from build123d import *

# Parameters (mm, degrees)
BASE_PROFILE_20MM_DEPTH   = 20
A_FRAME_BODY_200MM_DEPTH  = 200
FRAME_WINDOW_1_SKETCH_W   = 124.025088206
FRAME_WINDOW_1_SKETCH_H   = 160
FRAME_WINDOW_1_CUT_DEPTH  = 30
FRAME_WINDOW_2_SKETCH_W   = 43.365918468
FRAME_WINDOW_2_SKETCH_H   = 160
FRAME_WINDOW_2_CUT_DEPTH  = 30
THROUGH_OPENING_SKETCH_W  = 51.957421724
THROUGH_OPENING_SKETCH_H  = 25.341390787
THROUGH_OPENING_CUT_DEPTH = 200
WEB_BOSS_30MM_DEPTH       = 30
HUB_BOSS_30MM_DEPTH       = 30
HUB_BORE_SKETCH_R         = 25
HUB_BORE_CUT_DEPTH        = 120


with BuildPart() as part:
    # Base Profile Sketch → Base Profile 20mm (new body)
    with BuildSketch(Plane.XY):
        with BuildLine():
            Line((0, 200), (0, 0))
            Line((0, 0), (200, 0))
            Line((200, 0), (200, 20))
            Line((200, 20), (130, 20))
            ThreePointArc((130, 20), (122.928932188, 22.928932188), (120, 30))
            Line((120, 30), (120, 160))
            Line((120, 160), (120, 170))
            ThreePointArc((120, 170), (122.928932188, 177.071067812), (130, 180))
            Line((130, 180), (200, 180))
            Line((200, 180), (200, 200))
            Line((200, 200), (0, 200))
        make_face()
    extrude(amount=BASE_PROFILE_20MM_DEPTH)

    # Frame Profile Sketch → A-Frame Body 200mm (add)
    with BuildSketch(Plane.XZ):
        Polygon((120.794177907, 115.439301395), (94.123171193, 115.439301395), (91.530156651, 115.439301395), (48.56020139, 115.439301395), (0, 20), (24.280100695, 20), (59.946420611, 90.097910608), (111.903842335, 90.097910608), (174.506621983, 20), (200, 20), align=None)
    extrude(amount=-A_FRAME_BODY_200MM_DEPTH)

    # Frame Window 1 Sketch → Frame Window 1 Cut (cut)
    with BuildSketch(Plane(origin=(128.259685241, 0, 106.443715141), x_dir=(0.6386274199814919, 0, -0.7695160936899132), z_dir=(0.7695160936899134, 0, 0.6386274199814919))):
        with Locations((50.32261802, 100)):
            Rectangle(FRAME_WINDOW_1_SKETCH_W, FRAME_WINDOW_1_SKETCH_H)
    extrude(amount=-FRAME_WINDOW_1_CUT_DEPTH, mode=Mode.SUBTRACT)

    # Frame Window 2 Sketch → Frame Window 2 Cut (cut)
    with BuildSketch(Plane.XY.offset(115.439301395)):
        with Locations((99.111218673, 100)):
            Rectangle(FRAME_WINDOW_2_SKETCH_W, FRAME_WINDOW_2_SKETCH_H)
    extrude(amount=-FRAME_WINDOW_2_CUT_DEPTH, mode=Mode.SUBTRACT)

    # Through Opening Sketch → Through Opening Cut (cut)
    with BuildSketch(Plane.XZ):
        with Locations((85.925131473, 102.768606002)):
            Rectangle(THROUGH_OPENING_SKETCH_W, THROUGH_OPENING_SKETCH_H)
    extrude(amount=-THROUGH_OPENING_CUT_DEPTH, mode=Mode.SUBTRACT)

    # Web Sketch → Web Boss 30mm (add)
    with BuildSketch(Plane.XY.offset(115.439301395)):
        with BuildLine():
            Line((48.56020139, 200), (120.794177907, 200))
            Line((120.794177907, 200), (120.794177907, 180))
            Line((120.794177907, 180), (97.556604563, 180))
            ThreePointArc((97.556604563, 180), (90.485536751, 177.071067812), (87.556604563, 170))
            Line((87.556604563, 170), (87.556604563, 30))
            ThreePointArc((87.556604563, 30), (90.485536751, 22.928932188), (97.556604563, 20))
            Line((97.556604563, 20), (120.794177907, 20))
            Line((120.794177907, 20), (120.794177907, 0))
            Line((120.794177907, 0), (48.56020139, 0))
            Line((48.56020139, 0), (48.56020139, 200))
        make_face()
    extrude(amount=-WEB_BOSS_30MM_DEPTH)

    # Hub Boss Sketch → Hub Boss 30mm (add)
    with BuildSketch(Plane.XY.offset(115.439301395)):
        with BuildLine():
            Line((87.556604563, 145), (87.556604563, 55))
            ThreePointArc((87.556604563, 55), (132.556604563, 100), (87.556604563, 145))
        make_face()
    extrude(amount=-HUB_BOSS_30MM_DEPTH)

    # Hub Bore Sketch → Hub Bore Cut (cut)
    with BuildSketch(Plane.XY.offset(115.439301395)):
        with Locations((87.556604563, 100)):
            Circle(HUB_BORE_SKETCH_R)
    extrude(amount=-HUB_BORE_CUT_DEPTH, mode=Mode.SUBTRACT)


solid = part.part
Design review of the part built by this model. Coordinates are the model's own, in mm. A direction names the side the tool comes from. Give positions to 0.01 mm unless a question says otherwise; leave off trailing zeros. Order: outer loops, then holes, each group sorted by start corner. A loop starts at its lowest first (then second) coordinate and runs counter-clockwise, first axis right, second up.
1. Tool access review of faces 5 (the cylindrical face through (122.85, 176.99, 9.86)), 6 (the flat face through (120, 99, 10)), 7 (the cylindrical face through (67.717, 84.788, 100.649)), 8 (the flat face through (149, 180, 49)), 9 (the flat face through (121, 0, 84)): name each direction out of +Z, -Z, +X, -X, +Y, -Y from which nothing blocks a thin tool from reaching the whole face with its end or side.
Solution:
face 5: +Z, -Z, +X
face 6: -Z, +X
face 7: +Z, -Z
face 8: +Z, +X
face 9: +Z, -Z, +X, -X, -Y
2. To check wall thickness, follow L1, parallel to Z at x = 75, y = 10; L2, parallel to Y at x = 89, z = 87; L3, parallel to Y at x = 104.5, z = 14. State the ranges of each line that lie inside material, in increasing order.
Solution:
L1: z = 0 to 20, 85.44 to 115.44
L2: y = 0 to 24.82, 55.02 to 75.04, 124.96 to 144.98, 175.18 to 200
L3: y = 0 to 81.62, 118.38 to 200
3. Add section B-B, the plane x = 183.5. State the section outline as (y, z) points, then the cut area to 3 significant figures.
Solution:
outline: (0, 0) - (20, 0) - (20, 39.88) - (0, 39.88) - close; (180, 0) - (200, 0) - (200, 39.88) - (180, 39.88) - close
area: 1,600 mm2
4. Add section C-C, the plane y = 17. State the section outline as (x, z) points.
Solution:
outline: (0, 0) - (200, 0) - (200, 20) - (120.79, 115.44) - (48.56, 115.44) - (0, 20) - close; hole (24.28, 20) - (174.51, 20) - (116.06, 85.44) - (57.58, 85.44) - close
5. Mouldability with a two-part tool opening along Y and no side actions: class faces 1 (the flat face through (121, 200, 84)), 2 (the flat face through (54, 101, 0)), 3 (the flat face through (149, 20, 49)), 4 (the cylindrical face through (132.546, 99.01, 100.649)) as +Y half, -Y half, draft (parallel to the pull), parting line (faces both ways), or undercut.
Solution:
face 1: +Y half
face 2: draft
face 3: undercut
face 4: undercut
6. For pin 1 Ø16 at (y, z) = (66.5, 7) entering from +X; pin 2 Ø10 at (y, z) = (99, 103.5) entering from +X; pin 3 Ø12 at (x, z) = (162.5, 55.5) entering from -Y, all flat-tipped, find the tip position at first contact; note any pin that passes through.
Solution:
pin 1: stops at x = 120
pin 2: stops at x = 132.56
pin 3: stops at y = 0
7. Add section D-D, the plane z = 13. State the section outline as (x, y) points, then the cut area to 3 significant figures.
Solution:
outline: (0, 0) - (200, 0) - (200, 20) - (130, 20) arc R10 cw to (120, 30) - (120, 170) arc R10 cw to (130, 180) - (200, 180) - (200, 200) - (0, 200) - close; hole circle Ø50 at (87.56, 100)
area: 25,300 mm2
8. Add section A-A, the plane y = 100. State the section outline as (x, z) points, then the cut area to 3 significant figures.
Solution:
outline: (0, 0) - (62.56, 0) - (62.56, 20) - (24.28, 20) - (57.58, 85.44) - (62.56, 85.44) - (62.56, 115.44) - (48.56, 115.44) - (0, 20) - close; (112.56, 0) - (120, 0) - (120, 20) - (112.56, 20) - close; (112.56, 85.44) - (132.56, 85.44) - (132.56, 115.44) - (112.56, 115.44) - close
area: 4,240 mm2
